```python
from build123d import *

# Parameters (mm, degrees)
BOSS_EXTRUDE1_DEPTH = 20
CHAMFER1_SIZE       = 10


with BuildPart() as part:
    # Sketch1 → Boss-Extrude1 (new, symmetric)
    with BuildSketch(Plane(origin=(0, 0, 0), x_dir=(0, 0, -1), z_dir=(1, 0, 0))):
        with BuildLine():
            Line((0, 0), (0, 200))
            ThreePointArc((0, 200), (-28.284271247, 211.715728753), (-40, 240))
            Line((-40, 240), (-100, 240))
            Line((-100, 240), (-100, 200))
            Line((-100, 200), (-40, 0))
            Line((-40, 0), (0, 0))
        make_face()
    extrude(amount=BOSS_EXTRUDE1_DEPTH, both=True)

    # Chamfer1
    chamfer1_edges = [part.edges().sort_by_distance(p)[0] for p in [
        (20, 240, 70),
        (-20, 240, 70),
        (20, 100, 0),
        (-20, 100, 0),
    ]]
    chamfer(chamfer1_edges, length=CHAMFER1_SIZE)


solid = part.part
```
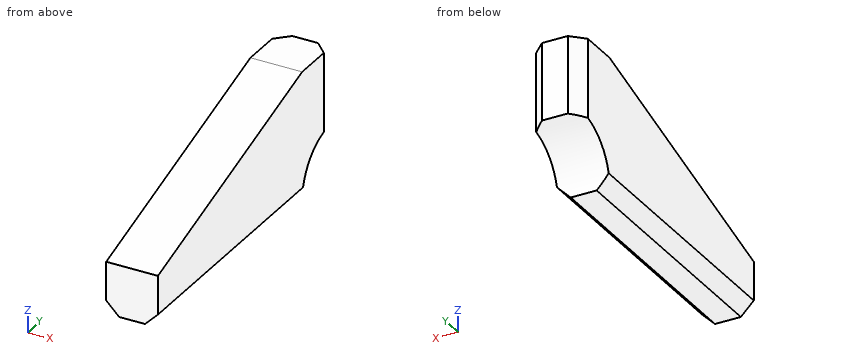
The model under review builds one solid part; all positions refer to its coordinate system, in mm. Round coordinates to 2 decimals unless told otherwise and drop trailing zeros. Loops run counter-clockwise (first coordinate to the right, second up) from the corner with the lowest first, then second, coordinate; pieces in that order, holes last. Notation, with made-up numbers: M 17,17.25 L 43,17.25 A7 cw 43,28.25 Z; hole C 89,-5.5 d4. An arc over 180 degrees is marked long. Put each result on its own line as item: value.
Q1. Consider section A-A, the plane y = 121. Give the boundary of the cut face in (x, z), then the cut area to 3 significant figures.
Result set:
outline: M -20,10 L -10,0 L 10,0 L 20,10 L 20,76.3 L -20,76.3 Z
area: 2,950 mm²
Q2. Consider section D-D, the plane y = 220.5. Give the boundary of the cut face in (x, z), then the cut area to 3 significant figures.
Result set:
outline: M -20,34.92 L 20,34.92 L 20,100 L -20,100 Z
area: 2,600 mm²
Q3. For pin 1 (4 mm diameter, centred on x = 12.5, y = 30.5, fed in from -Z), flat-tipped, find the tip position at first contact; note if it passes through.
Result set:
pin 1: stops at z = 0.5
Q4. Consider section C-C, the plane z = 26. Give the boundary of the cut face in (x, y), then the cut area to 3 significant figures.
Result set:
outline: M -20,0 L 20,0 L 20,209.6 L -20,209.6 Z
area: 8,380 mm²
Q5. To check wall thickness, follow L1, parallel to Z at x = 12, y = 195; L2, parallel to Z at x = 9, y = 185; L3, parallel to Y at x = 7.5, z = 5. State the ranges of each line that lie inside material, in increasing order.
Result set:
L1: z = 2 to 98.5
L2: z = 0 to 95.5
L3: y = 0 to 200.31
Q6. Consider section B-B, the plane z = 71.5. Give the boundary of the cut face in (x, y).
Result set:
outline: M -20,105 L 20,105 L 20,230 L 10,240 L -10,240 L -20,230 Z
